Model file for the job. Use its own axes, mm. A direction names the side the tool comes from. Round coordinates to 2 decimals unless told otherwise and drop trailing zeros. Loops run counter-clockwise (first coordinate to the right, second up) from the corner with the lowest first, then second, coordinate; pieces in that order, holes last. Notation, with made-up numbers: (-5.75, 89.5) -> (32.25, 89.5) arc R32 cw to (32.25, 123.5) -> close; hole circle Ø8 at (-22, -14.75). An arc over 180 degrees is marked (long way). Use a Markdown table: item, result.
from build123d import *

# Parameters (mm, degrees)
SKETCH_2_W                   = 90
SKETCH_2_H                   = 60
EXTRUDE_1_DEPTH              = 12
SKETCH_3_W                   = 2
SKETCH_3_H                   = 20
CUT_EXTRUDE_1_DEPTH          = 109.830142883
SKETCH_4_W                   = 10
SKETCH_4_H                   = 1
CUT_EXTRUDE_2_DEPTH          = 109.830142883
HOLE_WIZARD_M6_3_D           = 6.6
HOLE_WIZARD_M6_3_DEPTH       = 17
HOLE_WIZARD_M6_3_CBORE_D     = 11
HOLE_WIZARD_M6_3_CBORE_DEPTH = 6.4
HOLE_WIZARD_M6_3_TIP         = 1.982840043
CHAMFER_1_SIZE               = 2
HOLE_WIZARD_M3_1_D           = 2.5
HOLE_WIZARD_M3_1_DEPTH       = 8.5
HOLE_WIZARD_M3_1_TIP         = 0.751075774
SKETCH_15_W                  = 10
SKETCH_15_H                  = 60
EXTRUDE_2_DEPTH              = 44
SKETCH_16_W                  = 5
SKETCH_16_H                  = 60
CUT_EXTRUDE_3_DEPTH          = 117.400171821
HOLE_WIZARD_M6_1_D           = 5
HOLE_WIZARD_M6_1_DEPTH       = 17
HOLE_WIZARD_M6_1_TIP         = 1.502151548
CHAMFER_2_SIZE               = 2


with BuildPart() as part:
    # 草图2 → 凸台-拉伸1 (new body)
    with BuildSketch(Plane.XY):
        with Locations((45, -30)):
            Rectangle(SKETCH_2_W, SKETCH_2_H)
    extrude(amount=EXTRUDE_1_DEPTH)

    # 草图3 → 切除-拉伸1 (cut, through all)
    with BuildSketch(Plane(origin=(90, 0, 0), x_dir=(0, 0, -1), z_dir=(1, 0, 0))):
        with Locations((-11, -15)):
            Rectangle(SKETCH_3_W, SKETCH_3_H)
    extrude(amount=-CUT_EXTRUDE_1_DEPTH, mode=Mode.SUBTRACT)

    # 草图4 → 切除-拉伸2 (cut, through all)
    with BuildSketch(Plane(origin=(0, 0, 0), x_dir=(1, 0, 0), z_dir=(0, 1, 0))):
        with Locations((80, -0.5)):
            Rectangle(SKETCH_4_W, SKETCH_4_H)
    extrude(amount=-CUT_EXTRUDE_2_DEPTH, mode=Mode.SUBTRACT)

    # M6 六角凹头螺钉的柱形沉头孔3
    with Locations(Plane(origin=(0, 0, 0), x_dir=(-1, 0, 0), z_dir=(0, 0, -1))):
        with Locations((-60, -15), (-15, -15)):
            CounterBoreHole(HOLE_WIZARD_M6_3_D / 2, HOLE_WIZARD_M6_3_CBORE_D / 2, HOLE_WIZARD_M6_3_CBORE_DEPTH, depth=HOLE_WIZARD_M6_3_DEPTH)
            with Locations((0, 0, -(HOLE_WIZARD_M6_3_DEPTH + HOLE_WIZARD_M6_3_TIP / 2))):  # 118° drill point
                Cone(0, HOLE_WIZARD_M6_3_D / 2, HOLE_WIZARD_M6_3_TIP, mode=Mode.SUBTRACT)

    # 倒角1
    chamfer_1_edges = [part.edges().sort_by_distance(p)[0] for p in [
        (0, 0, 6),
        (90, 0, 6),
        (90, -60, 6),
        (0, -60, 6),
    ]]
    chamfer(chamfer_1_edges, length=CHAMFER_1_SIZE)

    # M3 螺纹孔1
    with Locations(Plane(origin=(0, -60, 0), x_dir=(-1, 0, 0), z_dir=(0, -1, 0))):
        with Locations((-70, -6)):
            Hole(HOLE_WIZARD_M3_1_D / 2, depth=HOLE_WIZARD_M3_1_DEPTH)
            with Locations((0, 0, -(HOLE_WIZARD_M3_1_DEPTH + HOLE_WIZARD_M3_1_TIP / 2))):  # 118° drill point
                Cone(0, HOLE_WIZARD_M3_1_D / 2, HOLE_WIZARD_M3_1_TIP, mode=Mode.SUBTRACT)

    # 草图15 → 凸台-拉伸2 (add)
    with BuildSketch(Plane(origin=(0, 0, 1), x_dir=(-1, 0, 0), z_dir=(0, 0, -1))):
        with Locations((-80, -30)):
            Rectangle(SKETCH_15_W, SKETCH_15_H)
    extrude(amount=EXTRUDE_2_DEPTH)

    # 草图16 → 切除-拉伸3 (cut, through all)
    with BuildSketch(Plane(origin=(0, 0, 0), x_dir=(-1, 0, 0), z_dir=(0, 0, -1))):
        with Locations((-87.5, -30)):
            Rectangle(SKETCH_16_W, SKETCH_16_H)
    extrude(amount=-CUT_EXTRUDE_3_DEPTH, mode=Mode.SUBTRACT)

    # M6 螺纹孔1
    with Locations(Plane(origin=(0, 0, -43), x_dir=(-1, 0, 0), z_dir=(0, 0, -1))):
        with Locations((-80, -15), (-80, -45)):
            Hole(HOLE_WIZARD_M6_1_D / 2, depth=HOLE_WIZARD_M6_1_DEPTH)
            with Locations((0, 0, -(HOLE_WIZARD_M6_1_DEPTH + HOLE_WIZARD_M6_1_TIP / 2))):  # 118° drill point
                Cone(0, HOLE_WIZARD_M6_1_D / 2, HOLE_WIZARD_M6_1_TIP, mode=Mode.SUBTRACT)

    # 倒角2
    chamfer_2_edges = [part.edges().sort_by_distance(p)[0] for p in [
        (80, -60, -43),
        (80, 0, -43),
    ]]
    chamfer(chamfer_2_edges, length=CHAMFER_2_SIZE)


solid = part.part
Q1. Tool access for faces 4 (the face through (37, -30, 0)), 5 (the face through (43, -5, 11)), 6 (the face through (65.495, -14.758, 3.155)), 7 (the face through (80, -1, -42)): list every direction of +Z, -Z, +X, -X, +Y, -Y with a clear straight run to the whole face (end or side of a thin tool).
Results list:
| item | result |
|---|---|
| face 4 | -Z, -X, +Y, -Y |
| face 5 | +Z, +X, -X |
| face 6 | -Z |
| face 7 | -Z, +X, -X, +Y |
Q2. Band-saw the part on C-C, the plane z = -35. Give the cut face in (x, y).
Results list:
| item | result |
|---|---|
| outline | (75, -60) -> (85, -60) -> (85, 0) -> (75, 0) -> close; hole circle Ø5 at (80, -45); hole circle Ø5 at (80, -15) |
Q3. Band-saw the part on B-B, the plane y = -54.5. Give the cut face in (x, z), plus the area to 3 significant figures.
Results list:
| item | result |
|---|---|
| outline | (0, 0) -> (75, 0) -> (75, -43) -> (85, -43) -> (85, 12) -> (0, 12) -> close; hole circle Ø2.5 at (70, 6) |
| area | 1,450 mm² |
Q4. Pull direction Y, two halves, no side cores. Call faces 1 (the face through (42, -2, 12)), 2 (the face through (1, -59, 6)), 3 (the face through (16.19, -20.37, 3.16)): released by +Y, released by -Y, zero draft, split by the parting line, or undercut.
Results list:
| item | result |
|---|---|
| face 1 | zero draft |
| face 2 | released by -Y |
| face 3 | undercut |
Q5. Band-saw the part on A-A, the plane x = 60. Give the cut face in (y, z), plus the area to 3 significant figures.
Results list:
| item | result |
|---|---|
| outline | (-60, 0) -> (-20.5, 0) -> (-20.5, 6.4) -> (-18.3, 6.4) -> (-18.3, 10) -> (-25, 10) -> (-25, 12) -> (-60, 12) -> close; (-11.7, 6.4) -> (-9.5, 6.4) -> (-9.5, 0) -> (0, 0) -> (0, 12) -> (-5, 12) -> (-5, 10) -> (-11.7, 10) -> close |
| area | 586 mm² |
Q6. Drill centre lines: L1, parallel to Y at x = 80, z = -37; L2, parallel to Y at x = 60, z = 7.55; L3, parallel to Y at x = 15, z = 1.75. Where is each one in solid material? Low to high. Write a range as from..to.
Results list:
| item | result |
|---|---|
| L1 | y = -60..-47.5, -42.5..-17.5, -12.5..0 |
| L2 | y = -60..-18.3, -11.7..0 |
| L3 | y = -60..-20.5, -9.5..0 |
Q7. Flat gauge pins, fed straight in: pin 1 (9 mm diameter, centred on x = 15, y = -15, fed in from +Z); pin 2 (3.5 mm diameter, centred on x = 17.5, y = -17, fed in from -Z); pin 3 (1.5 mm diameter, centred on x = 11.5, y = -34, fed in from -Z). Where does each tip first touch, or does it go through?
Results list:
| item | result |
|---|---|
| pin 1 | stops at z = 10 |
| pin 2 | stops at z = 6.4 |
| pin 3 | stops at z = 0 |
Q8. Band-saw the part on D-D, the plane x = 45.5. Give the cut face in (y, z).
Results list:
| item | result |
|---|---|
| outline | (-60, 0) -> (0, 0) -> (0, 12) -> (-5, 12) -> (-5, 10) -> (-25, 10) -> (-25, 12) -> (-60, 12) -> close |
